Can you work these out from the drawing? Everything is in mm from the part's minimum corner. A direction names the side the tool comes from. Coordinates: 2 decimals unless noted, no trailing zeros. Order: outer loops, then holes, each group sorted by start corner. A loop starts at its lowest first (then second) coordinate and runs counter-clockwise, first axis right, second up. Notation, with made-up numbers: (-10.75, 85) - (20.25, 85) arc R16 ccw to (20.25, 110) - close; hole circle Ø9 at (2.5, 13.5). An arc over 180 degrees is marked (long way). Answer as CSV lines item,"result". Start each with the question number.
Item 1: Imagine slicing it at D-D on y = 86.5. List the corners of the cut face in (x, z) for me, and give its area (3 significant figures).
Item 2: We'd pull the mould along Y, two halves only. Please class the marked faces 1, 2 and 3: pulls with the +Y half, pulls with the -Y half, needs draft (parallel to the pull), parting line crosses it, or undercut.
Item 3: Imagine slicing it at C-C on y = 38.5. List the corners of the cut face in (x, z) for me, and give its area (3 significant figures).
Item 4: Imagine slicing it at A-A on z = 59. List the corners of the cut face in (x, y) for me.
Item 5: I need wall thicknesses on line 1 (X direction, y = 72, z = 35); line 2 (Y direction, x = 9.5, z = 9); line 3 (Z direction, x = 62, y = 18). Which ranges of each line are inside material? Lowest first, please.
Item 6: Imagine slicing it at B-B on x = 87. List the corners of the cut face in (y, z) for me.
Item 7: On a 3-axis mill with a long thin cutter (end or side, diameter ignored), from which of +Z, -Z, +X, -X, +Y, -Y can I reach the whole of each face in a straight line? I mean the marked faces 4, 5, 6, 7 and 8. Say none if no direction works.
Item 8: I'm going to push flat-ended pins straight in: pin 1 (9.5 mm diameter, centred on x = 73, z = 7.5, fed in from +Y); pin 2 (5 mm diameter, centred on x = 30.5, z = 53, fed in from -Y); pin 3 (14.5 mm diameter, centred on x = 68, z = 44.5, fed in from +Y); pin 4 (2 mm diameter, centred on x = 102, y = 84.5, fed in from +Z). Where does each tip first touch, or does it pass through?
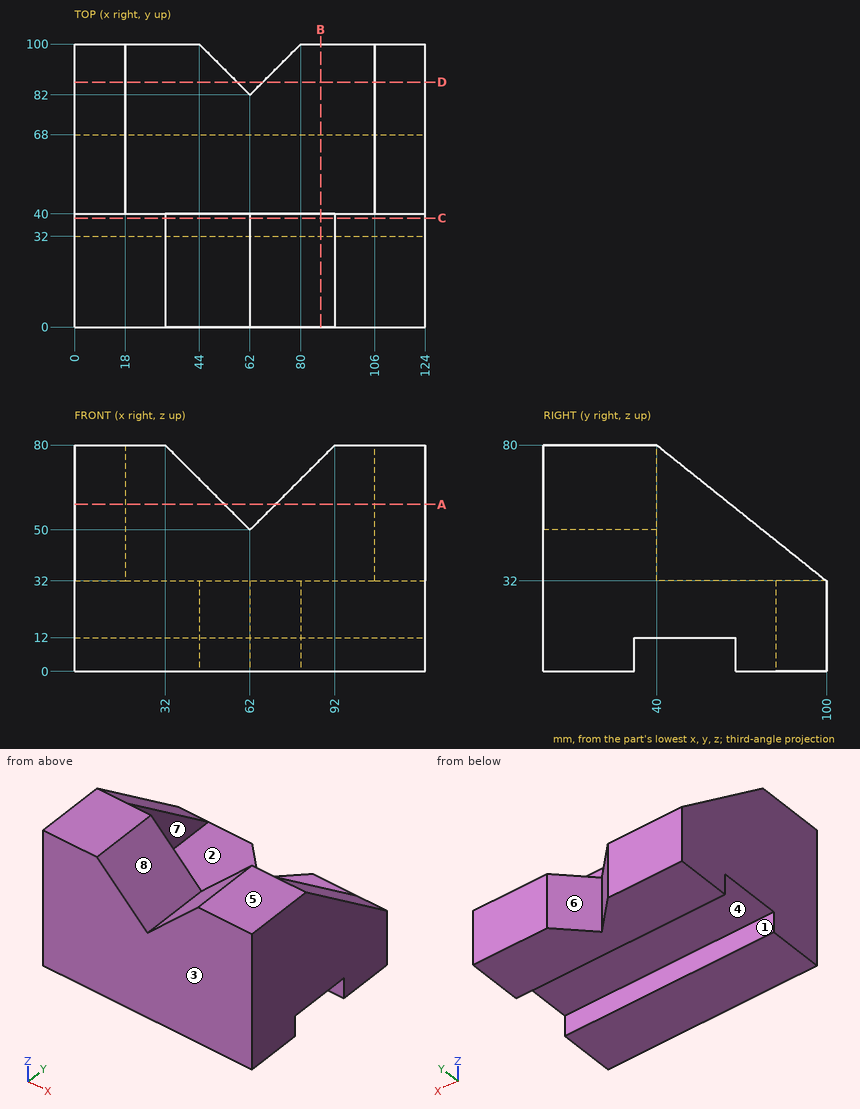
Responses:
1,outline,"(0, 0) - (57.5, 0) - (57.5, 32) - (18, 32) - (18, 42.8) - (0, 42.8) - close; (66.5, 0) - (124, 0) - (124, 42.8) - (106, 42.8) - (106, 32) - (66.5, 32) - close"
1,area,"4,070 mm^2"
2,face 1,"undercut"
2,face 2,"needs draft"
2,face 3,"pulls with the -Y half"
3,outline,"(0, 12) - (124, 12) - (124, 80) - (92, 80) - (62, 50) - (32, 80) - (0, 80) - close"
3,area,"7,530 mm^2"
4,outline,"(0, 0) - (53, 0) - (53, 40) - (18, 40) - (18, 66.25) - (0, 66.25) - close; (71, 0) - (124, 0) - (124, 66.25) - (106, 66.25) - (106, 40) - (71, 40) - close"
5,line 1,"x = 0 to 18, 106 to 124"
5,line 2,"y = 0 to 32, 68 to 100"
5,line 3,"z = 0 to 50"
6,outline,"(0, 0) - (32, 0) - (32, 12) - (68, 12) - (68, 0) - (100, 0) - (100, 32) - (40, 32) - (40, 75) - (0, 75) - close"
7,face 4,"-Z, +X, -X"
7,face 5,"+Z, +X, -X, +Y, -Y"
7,face 6,"+Z, -Z, +Y"
7,face 7,"+Z, +Y"
7,face 8,"+Z, +Y, -Y"
8,pin 1,"stops at y = 97.75"
8,pin 2,"stops at y = 0"
8,pin 3,"stops at y = 40"
8,pin 4,"stops at z = 32"
